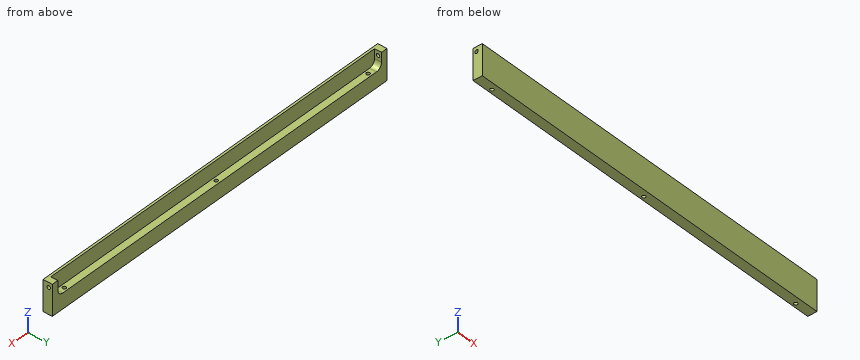
from build123d import *

# Parameters (mm, degrees)
SKETCH1_W                 = 670
SKETCH1_H                 = 52.68545994
BOSS_EXTRUDE1_DEPTH       = 16
SKETCH3_W                 = 648
SKETCH3_H                 = 81.022530329
CUT_EXTRUDE2_DEPTH        = 12
FILLET1_R                 = 10
F_6_0MM_DOWEL_HOLE1_D     = 6
F_6_0MM_DOWEL_HOLE1_DEPTH = 11
F_6_0MM_DOWEL_HOLE2_D     = 6


with BuildPart() as part:
    # Sketch1 → Boss-Extrude1 (new body)
    with BuildSketch(Plane(origin=(0, 0, 0), x_dir=(1, 0, 0), z_dir=(0, 1, 0))):
        Rectangle(SKETCH1_W, SKETCH1_H)
    extrude(amount=BOSS_EXTRUDE1_DEPTH)

    # Sketch3 → Cut-Extrude2 (cut)
    with BuildSketch(Plane(origin=(0, 16, 0), x_dir=(1, 0, 0), z_dir=(0, 1, 0))):
        with Locations((0, -40.511265165)):
            Rectangle(SKETCH3_W, SKETCH3_H)
    extrude(amount=-CUT_EXTRUDE2_DEPTH, mode=Mode.SUBTRACT)

    # Fillet1
    fillet1_edges = [part.edges().sort_by_distance(p)[0] for p in [
        (324, 10, 0),
        (-324, 10, 0),
    ]]
    fillet(fillet1_edges, radius=FILLET1_R)

    # Ø6.0mm Dowel Hole1
    with Locations(Plane.ZY.offset(-324)):
        with Locations((18.171364985, 10)):
            f_6_0mm_dowel_hole1 = Hole(F_6_0MM_DOWEL_HOLE1_D / 2, depth=F_6_0MM_DOWEL_HOLE1_DEPTH)

    # Mirror1: Ø6.0mm Dowel Hole1 across plane
    add(f_6_0mm_dowel_hole1.mirror(Plane(origin=(0, 0, 0), x_dir=(0, 0, 1), z_dir=(1, 0, 0))), mode=Mode.SUBTRACT)

    # Ø6.0mm Dowel Hole2 (through all)
    with Locations(Plane.XY):
        with Locations((304, 10), (0, 10)):
            f_6_0mm_dowel_hole2 = Hole(F_6_0MM_DOWEL_HOLE2_D / 2)

    # Mirror2: Ø6.0mm Dowel Hole2 across plane
    add(f_6_0mm_dowel_hole2.mirror(Plane(origin=(0, 0, 0), x_dir=(0, 0, 1), z_dir=(1, 0, 0))), mode=Mode.SUBTRACT)


solid = part.part
Could you check a few things on this model? Use its own coordinates, in mm. Give positions to 0.01 mm unless a question says otherwise; leave off trailing zeros. Answer as CSV lines item,"result". Start each with the question number.
(1) I'm going to push flat-ended pins straight in: pin 1 Ø2 at (x, z) = (-22, 6.5) entering from +Y; pin 2 Ø6 at (x, y) = (92.5, 13) entering from +Z. Where does each tip first touch, or does it pass through?
(2) If we section it at A-A, the plane y = 10: Give the number of separate pieces and of enclosed holes in the cut face, and give its area (3 significant figures).
(3) Please list where these lines run through material, in increasing order: line 1 (X direction, y = 9.25, z = -7); line 2 (X direction, y = 6.5, z = 21.5); line 3 (X direction, y = 11.75, z = -15).
Answer list:
1,pin 1,"y = 4"
1,pin 2,"z = 0"
2,separate pieces,"6"
2,enclosed holes,"0"
2,area,"17,700 mm^2"
3,line 1,"-335 to -306.9, -301.1 to -2.9, 2.9 to 301.1, 306.9 to 335"
3,line 2,"-335 to -324, 324 to 335"
3,line 3,"-335 to -306.44, -301.56 to -2.44, 2.44 to 301.56, 306.44 to 335"
